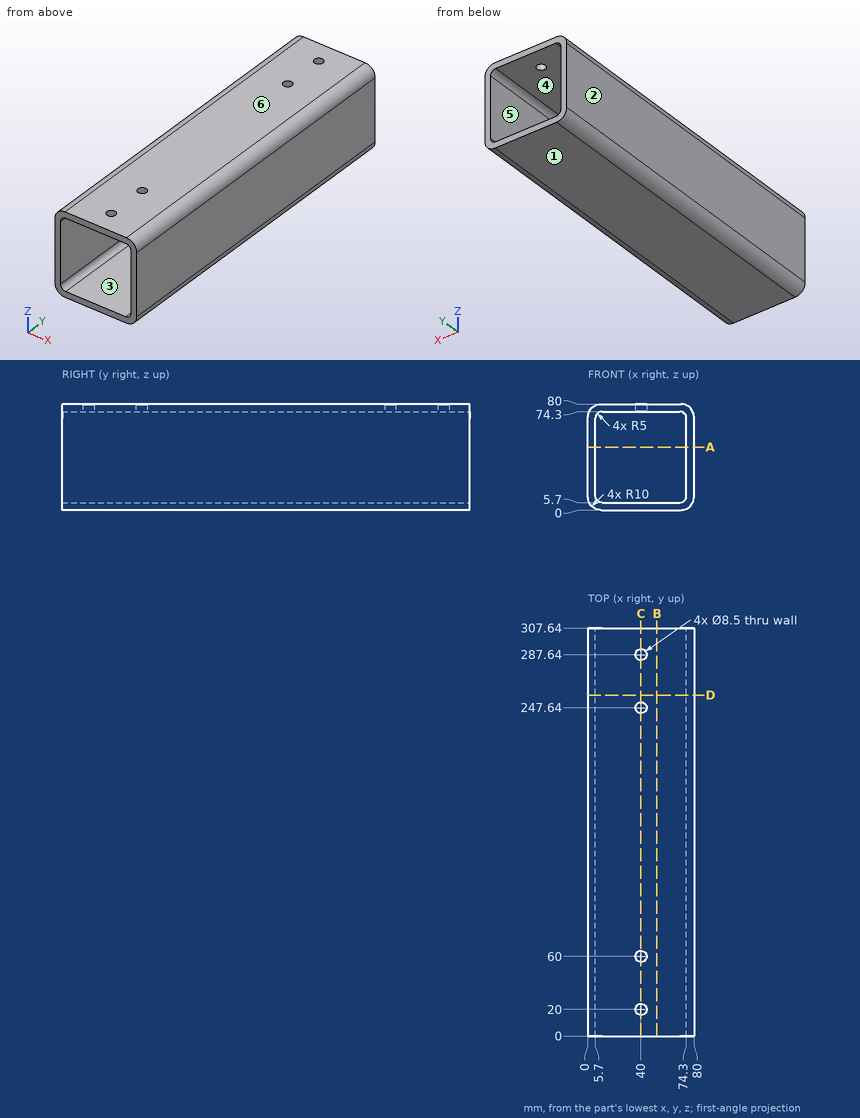
Verification items for this drawing (mm, ordinates from the low corner). A direction names the side the tool comes from. Give positions to 0.01 mm unless a question says otherwise; leave off trailing zeros. Order: outer loops, then holes, each group sorted by start corner. A loop starts at its lowest first (then second) coordinate and runs counter-clockwise, first axis right, second up. Notation, with made-up numbers: M 81,44.5 L 96,44.5 A17 ccw 96,57.5 Z; hole C -20.5,45 d2. An arc over 180 degrees is marked long. Use a Markdown table: item, result.
Item 1: Material ranges on line 1 along Y through (x, z) = (40, 75); line 2 along Z through (x, y) = (35, 153.5), recorded low to high.
Answers follow:
| item | result |
|---|---|
| line 1 | y = 0 to 15.75, 24.25 to 55.75, 64.25 to 243.39, 251.89 to 283.39, 291.89 to 307.64 |
| line 2 | z = 0 to 5.7, 74.3 to 80 |
Item 2: Section check D-D (y = 257). Record the cut outline in (x, z).
Answers follow:
| item | result |
|---|---|
| outline | M 0,10 A10 ccw 10,0 L 70,0 A10 ccw 80,10 L 80,70 A10 ccw 70,80 L 10,80 A10 ccw 0,70 Z; hole M 5.7,10.7 A5 ccw 10.7,5.7 L 69.3,5.7 A5 ccw 74.3,10.7 L 74.3,69.3 A5 ccw 69.3,74.3 L 10.7,74.3 A5 ccw 5.7,69.3 Z |
Item 3: Section check C-C (x = 40). Record the cut outline in (y, z).
Answers follow:
| item | result |
|---|---|
| outline | M 0,0 L 307.64,0 L 307.64,5.7 L 0,5.7 Z; M 0,74.3 L 15.75,74.3 L 15.75,80 L 0,80 Z; M 24.25,74.3 L 55.75,74.3 L 55.75,80 L 24.25,80 Z; M 64.25,74.3 L 243.39,74.3 L 243.39,80 L 64.25,80 Z; M 251.89,74.3 L 283.39,74.3 L 283.39,80 L 251.89,80 Z; M 291.89,74.3 L 307.64,74.3 L 307.64,80 L 291.89,80 Z |
Item 4: Section check B-B (x = 52). Record the cut outline in (y, z).
Answers follow:
| item | result |
|---|---|
| outline | M 0,0 L 307.64,0 L 307.64,5.7 L 0,5.7 Z; M 0,74.3 L 307.64,74.3 L 307.64,80 L 0,80 Z |
Item 5: Tool access check on the marked faces 5 and 6. Record the directions out of +Z, -Z, +X, -X, +Y, -Y that give a thin tool (end or side, any length) a straight path to the whole face; none if there is none.
Answers follow:
| item | result |
|---|---|
| face 5 | +Y, -Y |
| face 6 | +Z, +X, -X, +Y, -Y |
Item 6: Draft check along X on the marked faces 1, 2, 3 and 4. Enter one of: +X half, -X half, draft (parallel to the pull), parting line (faces both ways), or undercut.
Answers follow:
| item | result |
|---|---|
| face 1 | draft |
| face 2 | -X half |
| face 3 | undercut |
| face 4 | undercut |
Item 7: Section check A-A (z = 47.5). Record the cut outline in (x, y).
Answers follow:
| item | result |
|---|---|
| outline | M 0,0 L 5.7,0 L 5.7,307.64 L 0,307.64 Z; M 74.3,0 L 80,0 L 80,307.64 L 74.3,307.64 Z |
